Verification items for the finished model (mm, model axes). A direction names the side the tool comes from. Give positions to 0.01 mm unless a question says otherwise; leave off trailing zeros. Order: outer loops, then holes, each group sorted by start corner. A loop starts at its lowest first (then second) coordinate and runs counter-clockwise, first axis right, second up.
(1) Mould release check, pull along Z, two halves, no side actions. Record for faces 1 (the face through (-192.617, 18.34, 17.22)), 2 (the face through (-196.561, 7.509, 23.846)), 3 (the face through (-200.617, 22.9, 10.4)), 4 (the face through (513.587, -14.418, 45.783)): pulls with the +Z half, pulls with the -Z half, needs draft (parallel to the pull), parting line crosses it, or undercut.
(2) Gauge pin test, flat ends, axial feed: pin 1 (1.5 mm diameter, centred on x = 3.5, z = -14.5, fed in from +Y); pin 2 (3 mm diameter, centred on x = 262.5, y = -27.5, fed in from -Z); pin 3 (5 mm diameter, centred on x = 296.5, z = -19.5, fed in from +Y). Record the tip position at first contact, or that the pin passes through.
(3) Scan lines: L1, parallel to Z at x = 44, y = 0; L2, parallel to Y at x = -197, z = 0. Record each from-to range of solid material in increasing order.
(4) Sectioned sample at A-A on y = 0. Record the cut outline in (x, z), plus the area to 3 significant figures.
(5) Sectioned sample at C-C on x = 316. Record the cut outline in (y, z).
(6) Sectioned sample at D-D on z = -33. Record the cut outline in (x, y).
(7) Access from +Z, -Z, +X, -X, +Y, -Y to the whole of each face (thin tool, end or side, straight path). Record for faces 5 (the face through (164.94, -39.05, -8.67)), 6 (the face through (509.643, -19, 45)), 7 (the face through (525.04, -15.02, 47.69)).
```python
from build123d import *

# Parameters (mm, degrees)
EXTRUDE_START   = 200
SKETCH_3_R      = 50
SKETCH_3_R_2    = 40
EXTRUDE_1_DEPTH = 200
EXTRUDE_START_2 = -8
SKETCH_4_R      = 40
SKETCH_4_R_2    = 25
EXTRUDE_2_DEPTH = 8


with BuildPart() as part:
    # 草图2 → 旋转1 (revolve)
    with BuildSketch(Plane.XY, mode=Mode.PRIVATE) as revolve_1_sk:
        Polygon((-22.357142857, 40), (532.642857143, 40), (532.642857143, 50), (517.642857143, 50), (517.642857143, 48), (509.642857143, 48), (509.642857143, 50), (-0.617142857, 50), (-0.617142857, 48), (-8.617142857, 48), (-8.617142857, 50), (-22.357142857, 50), align=None)
    revolve(revolve_1_sk.sketch.rotate(Axis((-27.214285714, 0, 0), (1, 0, 0)), 90), axis=Axis((-27.214285714, 0, 0), (1, 0, 0)))

    # 草图3 → 凸台-拉伸1 (add)
    with BuildSketch(Plane.ZY.offset(0.617142857).offset(EXTRUDE_START)):
        Circle(SKETCH_3_R)
        Circle(SKETCH_3_R_2, mode=Mode.SUBTRACT)
    extrude(amount=-EXTRUDE_1_DEPTH)

    # 草图4 → 凸台-拉伸2 (add)
    with BuildSketch(Plane.ZY.offset(200.617142857).offset(EXTRUDE_START_2)):
        Circle(SKETCH_4_R)
        Circle(SKETCH_4_R_2, mode=Mode.SUBTRACT)
    extrude(amount=EXTRUDE_2_DEPTH)


solid = part.part
```
Ans:
1. face 1: undercut
1. face 2: undercut
1. face 3: needs draft
1. face 4: parting line crosses it
2. pin 1: stops at y = 48.07
2. pin 2: stops at z = -42.71
2. pin 3: stops at y = 47.02
3. L1: z = -50 to -40, 40 to 50
3. L2: y = -50 to -25, 25 to 50
4. outline: (-200.62, -50) - (509.64, -50) - (509.64, -48) - (517.64, -48) - (517.64, -50) - (532.64, -50) - (532.64, -40) - (-192.62, -40) - (-192.62, -25) - (-200.62, -25) - close; (-200.62, 25) - (-192.62, 25) - (-192.62, 40) - (532.64, 40) - (532.64, 50) - (517.64, 50) - (517.64, 48) - (509.64, 48) - (509.64, 50) - (-200.62, 50) - close
4. area: 14,900 mm2
5. outline: circle Ø100 at (0, 0); hole circle Ø80 at (0, 0)
6. outline: (-200.62, -37.56) - (509.64, -37.56) - (509.64, -34.86) - (517.64, -34.86) - (517.64, -37.56) - (532.64, -37.56) - (532.64, -22.61) - (-192.62, -22.61) - (-192.62, 22.61) - (532.64, 22.61) - (532.64, 37.56) - (517.64, 37.56) - (517.64, 34.86) - (509.64, 34.86) - (509.64, 37.56) - (-200.62, 37.56) - close
7. face 5: +X
7. face 6: none
7. face 7: +X, -X
